from build123d import *

# Parameters (mm, degrees)
BACK_PLATE_DEPTH        = 10
MOUNTING_HOLES_SKETCH_R = 4.5
MOUNTING_HOLES_2X_DEPTH = 10
L_BASE_BODY_DEPTH       = 64
HUB_BOSS_SKETCH_R       = 12
HUB_BOSS_DEPTH          = 10
SUPPORT_RIB_DEPTH       = 5
HUB_BORE_SKETCH_R       = 8
HUB_BORE_16_DEPTH       = 30
FRONT_SLOT_DEPTH        = 30
EDGE_FILLET_R10_A_R     = 10
EDGE_FILLET_R10_B_R     = 10


with BuildPart() as part:
    # Back Plate Sketch → Back Plate (new body)
    with BuildSketch(Plane.XY):
        with BuildLine():
            Line((0, 0), (0, 41))
            ThreePointArc((0, 41), (2.636038969, 47.363961031), (9, 50))
            Line((9, 50), (55, 50))
            ThreePointArc((55, 50), (61.363961031, 47.363961031), (64, 41))
            Line((64, 41), (64, 0))
            Line((64, 0), (0, 0))
        make_face()
    extrude(amount=BACK_PLATE_DEPTH)

    # Mounting Holes Sketch → Mounting Holes 2x (cut)
    with BuildSketch(Plane.XY.offset(10)):
        with Locations((9, 41)):
            Circle(MOUNTING_HOLES_SKETCH_R)
        with Locations((55, 41)):
            Circle(MOUNTING_HOLES_SKETCH_R)
    extrude(amount=-MOUNTING_HOLES_2X_DEPTH, mode=Mode.SUBTRACT)

    # L-Base Profile Sketch → L-Base Body (add)
    with BuildSketch(Plane.ZY):
        Polygon((0, 0), (39, 0), (39, 3), (60, 3), (60, -28), (69, -28), (69, 12), (0, 12), align=None)
    extrude(amount=-L_BASE_BODY_DEPTH)



with BuildPart() as body_2:
    # Hub Boss Sketch → Hub Boss (new, symmetric)
    with BuildSketch(Plane.ZY.offset(-32)):
        with Locations((37, 32)):
            Circle(HUB_BOSS_SKETCH_R)
    extrude(amount=HUB_BOSS_DEPTH, both=True)


with BuildPart() as part_1:
    add(part.part)

    add(body_2.part)  # Support Rib merges body 2
    # Support Rib Sketch → Support Rib (add, symmetric)
    with BuildSketch(Plane.ZY.offset(-32)):
        with BuildLine():
            Line((10, 12), (69, 12))
            Line((69, 12), (44.830635443, 41.092917494))
            Line((44.830635443, 41.092917494), (35.339623776, 43.884576172))
            Line((35.339623776, 43.884576172), (12.426606273, 47.573393727))
            ThreePointArc((12.426606273, 47.573393727), (10.710736522, 48.284130249), (10, 50))
            Line((10, 50), (10, 12))
        make_face()
    extrude(amount=SUPPORT_RIB_DEPTH, both=True)

    # Hub Bore Sketch → Hub Bore Ø16 (cut, symmetric)
    with BuildSketch(Plane.ZY.offset(-22)):
        with Locations((37, 32)):
            Circle(HUB_BORE_SKETCH_R)
    extrude(amount=HUB_BORE_16_DEPTH, both=True, mode=Mode.SUBTRACT)

    # Front Slot Sketch → Front Slot (cut, symmetric)
    with BuildSketch(Plane.XY.offset(69)):
        with BuildLine():
            Line((23, -15.5), (41, -15.5))
            ThreePointArc((41, -15.5), (43.5, -18), (41, -20.5))
            Line((41, -20.5), (23, -20.5))
            ThreePointArc((23, -20.5), (20.5, -18), (23, -15.5))
        make_face()
    extrude(amount=FRONT_SLOT_DEPTH, both=True, mode=Mode.SUBTRACT)

    # Edge Fillet R10 A
    edge_fillet_r10_a_edges = [part_1.edges().sort_by_distance(p)[0] for p in [
        (0, -28, 64.5),
    ]]
    fillet(edge_fillet_r10_a_edges, radius=EDGE_FILLET_R10_A_R)

    # Edge Fillet R10 B
    edge_fillet_r10_b_edges = [part_1.edges().sort_by_distance(p)[0] for p in [
        (64, -28, 64.5),
    ]]
    fillet(edge_fillet_r10_b_edges, radius=EDGE_FILLET_R10_B_R)


solid = part_1.part
Source: CAD feature listing. Evaluate the final solid. Frame: model axes, mm. A direction names the side the tool comes from. Coordinates: 2 decimals unless noted, no trailing zeros. Order: outer loops, then holes, each group sorted by start corner. A loop starts at its lowest first (then second) coordinate and runs counter-clockwise, first axis right, second up.
Item 1: Cut plane A-A (z = 37). Return loops of the section in (x, y).
Output values:
outline: (0, 0) - (64, 0) - (64, 12) - (37, 12) - (37, 20) - (42, 20) - (42, 24) - (22, 24) - (22, 20) - (27, 20) - (27, 12) - (0, 12) - close; (22, 40) - (42, 40) - (42, 44) - (22, 44) - close
Item 2: Cut plane B-B (y = 32). Return loops of the section in (x, z), plus the area to 3 significant figures.
Output values:
outline: (0, 0) - (64, 0) - (64, 10) - (37, 10) - (37, 25) - (42, 25) - (42, 29) - (22, 29) - (22, 25) - (27, 25) - (27, 10) - (0, 10) - close; (22, 45) - (42, 45) - (42, 49) - (37, 49) - (37, 52.38) - (27, 52.38) - (27, 49) - (22, 49) - close
area: 984 mm2
Item 3: First-contact query: P1, Ø5, axis at y = 18.5, z = 46.5, coming from the +X side; P2, Ø1, axis at x = 18.5, z = 38, coming from the +Y side; P3, Ø19, axis at y = 31, z = 37, coming from the -X side; P4, Ø5.5, axis at x = 55, y = 41, coming from the -Z side. Flat tips, straight axial feed; report the tip coordinate or a pass-through.
Output values:
P1: stops at x = 37
P2: stops at y = 12
P3: stops at x = 22
P4: passes through
Item 4: Set-up query: faces 1 (the face through (22, 24, 39)), 2 (the face through (32, 1, 39)), 3 (the face through (32, -20.5, 65)), 4 (the face through (32, 0, 19)). Return all of +Z, -Z, +X, -X, +Y, -Y with unobstructed straight access to the full face (end or side cutting, diameter ignored); none if empty.
Output values:
face 1: +Z, -X, +Y
face 2: +X, -X, -Y
face 3: +Z, -Z
face 4: -Z, +X, -X, -Y
Item 5: Material intervals for line 1 (Y direction, x = 30.75, z = 37); line 2 (Y direction, x = 9, z = 4.25); line 3 (Y direction, x = 40, z = 20.5), sorted ascending.
Output values:
line 1: y = 0 to 24, 40 to 44
line 2: y = 0 to 36.5, 45.5 to 50
line 3: y = 0 to 12
Item 6: Pull-direction query (Z, two-part tool) for faces 5 (the face through (31.93, 48.265, 10.73)), 6 (the face through (32, 3, 49)), 7 (the face through (0, 9, 27)); classes: pulls with the +Z half, pulls with the -Z half, needs draft (parallel to the pull), parting line crosses it, or undercut.
Output values:
face 5: pulls with the +Z half
face 6: undercut
face 7: needs draft
Item 7: Cut plane C-C (x = 47). Return loops of the section in (y, z), plus the area to 3 significant figures.
Output values:
outline: (-28, 60) - (3, 60) - (3, 39) - (0, 39) - (0, 0) - (50, 0) - (50, 10) - (12, 10) - (12, 69) - (-28, 69) - close
area: 1,400 mm2
Item 8: Cut plane D-D (z = 53). Return loops of the section in (x, y), plus the area to 3 significant figures.
Output values:
outline: (0, 3) - (64, 3) - (64, 12) - (37, 12) - (37, 31.26) - (27, 31.26) - (27, 12) - (0, 12) - close
area: 769 mm2
